Verification items for the finished model (mm, model axes). Face numbers are marked on the shaded views. Coordinates: 2 decimals unless noted, no trailing zeros. Write each loop counter-clockwise with the first axis right and the second up, starting at its lowest first coordinate (ties: lowest second). Pieces come first, ordered by that corner, then holes. Notation, with made-up numbers: (63.25, 73.5) -> (73.25, 73.5) arc R25 ccw to (73.25, 103.5) -> close; hole circle Ø1 at (65, 75). An arc over 180 degrees is marked (long way). Answer in a Markdown table with one row per item.
```python
from build123d import *

# Parameters (mm, degrees)
SKETCH_1_W                = 30
SKETCH_1_H                = 62
EXTRUDE_1_DEPTH           = 12
SKETCH_2_W                = 22.1
SKETCH_2_H                = 56.1
CUT_EXTRUDE_1_DEPTH       = 2
SKETCH_3_W                = 3
SKETCH_3_H                = 72.139143417
CUT_EXTRUDE_2_DEPTH       = 2
SKETCH_4_W                = 86.092630608
SKETCH_4_H                = 58.1
CUT_EXTRUDE_3_DEPTH       = 2
HOLE_WIZARD_M4_1_D        = 3.3
HOLE_WIZARD_1_D           = 4.5
HOLE_WIZARD_1_CBORE_D     = 8
HOLE_WIZARD_1_CBORE_DEPTH = 5
CHAMFER_1_SIZE            = 1


with BuildPart() as part:
    # 草图1 → 凸台-拉伸1 (new body)
    with BuildSketch(Plane(origin=(0, 0, 0), x_dir=(1, 0, 0), z_dir=(0, 1, 0))):
        Rectangle(SKETCH_1_W, SKETCH_1_H)
    extrude(amount=EXTRUDE_1_DEPTH)

    # 草图2 → 切除-拉伸1 (cut)
    with BuildSketch(Plane.XZ):
        Rectangle(SKETCH_2_W, SKETCH_2_H)
    extrude(amount=-CUT_EXTRUDE_1_DEPTH, mode=Mode.SUBTRACT)

    # 草图3 → 切除-拉伸2 (cut)
    with BuildSketch(Plane.XZ):
        with Locations((-9.55, 0.756704302)):
            Rectangle(SKETCH_3_W, SKETCH_3_H)
    cut_extrude_2 = extrude(amount=-CUT_EXTRUDE_2_DEPTH, mode=Mode.SUBTRACT)

    # 镜向1: 切除-拉伸2 across plane
    add(cut_extrude_2.mirror(Plane(origin=(0, 0, 0), x_dir=(0, 0, 1), z_dir=(1, 0, 0))), mode=Mode.SUBTRACT)

    # 草图4 → 切除-拉伸3 (cut)
    with BuildSketch(Plane(origin=(0, 12, 0), x_dir=(1, 0, 0), z_dir=(0, 1, 0))):
        Rectangle(SKETCH_4_W, SKETCH_4_H)
    extrude(amount=-CUT_EXTRUDE_3_DEPTH, mode=Mode.SUBTRACT)

    # M4 螺纹孔1 (through all)
    with Locations(Plane(origin=(0, 10, 0), x_dir=(1, 0, 0), z_dir=(0, 1, 0))):
        with Locations((-10, 11.5), (10, 11.5), (-10, -11.5), (10, -11.5)):
            Hole(HOLE_WIZARD_M4_1_D / 2)

    # 打孔尺寸(%根据)开槽圆柱头螺钉的类型1 (through all)
    with Locations(Plane(origin=(0, 12, 0), x_dir=(1, 0, 0), z_dir=(0, 1, 0))):
        with Locations((-7, 24), (7, 24), (-7, -24), (7, -24)):
            CounterBoreHole(HOLE_WIZARD_1_D / 2, HOLE_WIZARD_1_CBORE_D / 2, HOLE_WIZARD_1_CBORE_DEPTH)

    # 倒角1
    chamfer_1_edges = [part.edges().sort_by_distance(p)[0] for p in [
        (15, 6, 31),
        (-15, 6, 31),
        (-15, 6, -31),
        (15, 6, -31),
    ]]
    chamfer(chamfer_1_edges, length=CHAMFER_1_SIZE)


solid = part.part
```
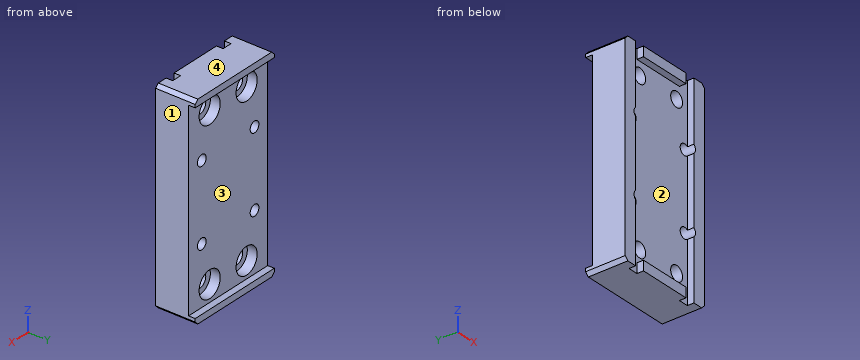
1. Sectioned sample at C-C, the plane y = 4.5. Count the separate pieces of the cut face and the enclosed holes in it, and give its area (3 significant figures).
Findings below:
| item | result |
|---|---|
| separate pieces | 1 |
| enclosed holes | 8 |
| area | 1,760 mm² |
2. Sectioned sample at A-A, the plane x = 7. Record the cut outline in (y, z), and give its area (3 significant figures).
Findings below:
| item | result |
|---|---|
| outline | (0, -31) -> (12, -31) -> (12, -29.05) -> (10, -29.05) -> (10, -28) -> (7, -28) -> (7, -26.25) -> (2, -26.25) -> (2, -28.05) -> (0, -28.05) -> close; (0, 28.05) -> (2, 28.05) -> (2, 26.25) -> (7, 26.25) -> (7, 28) -> (10, 28) -> (10, 29.05) -> (12, 29.05) -> (12, 31) -> (0, 31) -> close; (2, -21.75) -> (7, -21.75) -> (7, -20) -> (10, -20) -> (10, 20) -> (7, 20) -> (7, 21.75) -> (2, 21.75) -> close |
| area | 423 mm² |
3. Material ranges on probe 1 along X at (y, z) = (3.6, -24); probe 2 along X at (y, z) = (4, 11.5); probe 3 along Z at (x, y) = (-7, 4.9), recorded low to high. Write a range as from..to.
Findings below:
| item | result |
|---|---|
| probe 1 | x = -15..-9.25, -4.75..4.75, 9.25..15 |
| probe 2 | x = -15..-11.65, -8.35..8.35, 11.65..15 |
| probe 3 | z = -31..-26.25, -21.75..21.75, 26.25..31 |
4. Sectioned sample at B-B, the plane z = -24. Record the cut outline in (x, y).
Findings below:
| item | result |
|---|---|
| outline | (-15, 0) -> (-11.05, 0) -> (-11.05, 2) -> (-9.25, 2) -> (-9.25, 7) -> (-11, 7) -> (-11, 10) -> (-15, 10) -> close; (-4.75, 2) -> (4.75, 2) -> (4.75, 7) -> (3, 7) -> (3, 10) -> (-3, 10) -> (-3, 7) -> (-4.75, 7) -> close; (9.25, 2) -> (11.05, 2) -> (11.05, 0) -> (15, 0) -> (15, 10) -> (11, 10) -> (11, 7) -> (9.25, 7) -> close |
5. Sectioned sample at D-D, the plane x = -0.75. Record the cut outline in (y, z), and give its area (3 significant figures).
Findings below:
| item | result |
|---|---|
| outline | (0, -31) -> (12, -31) -> (12, -29.05) -> (10, -29.05) -> (10, 29.05) -> (12, 29.05) -> (12, 31) -> (0, 31) -> (0, 28.05) -> (2, 28.05) -> (2, -28.05) -> (0, -28.05) -> close |
| area | 516 mm² |
6. Go/stop test with flat-tipped pins: pin 1 (8 mm diameter, centred on x = -6, z = 16, fed in from -Y); pin 2 (2.5 mm diameter, centred on x = 10, z = -11.5, fed in from +Y); pin 3 (6.5 mm diameter, centred on x = 7, z = 24, fed in from +Y); pin 4 (4.5 mm diameter, centred on x = -10, z = -11.5, fed in from +Y). Record where each tip stops, or that it passes through.
Findings below:
| item | result |
|---|---|
| pin 1 | stops at y = 2 |
| pin 2 | passes through |
| pin 3 | stops at y = 7 |
| pin 4 | stops at y = 10 |
7. Release check for a two-part mould opening along Z. For the marked faces 1, 2, 3 and 4 record: released by +Z, released by -Z, zero draft, split by the parting line, or undercut.
Findings below:
| item | result |
|---|---|
| face 1 | zero draft |
| face 2 | undercut |
| face 3 | undercut |
| face 4 | released by +Z |
